Model file for the job. Use its own axes, mm. Round coordinates to 2 decimals unless told otherwise and drop trailing zeros. Order: outer loops, then holes, each group sorted by start corner. A loop starts at its lowest first (then second) coordinate and runs counter-clockwise, first axis right, second up. Notation, with made-up numbers: (-14.75, 75) -> (38.25, 75) arc R22 cw to (38.25, 102) -> close; hole circle Ø4 at (52, 87). An arc over 180 degrees is marked (long way). Answer as CSV lines item,"result".
```python
from build123d import *

# Parameters (mm, degrees)
SKETCH1_W           = 139.7
SKETCH1_H           = 38.1
SKETCH1_R           = 7.1374
BOSS_EXTRUDE1_DEPTH = 4


with BuildPart() as part:
    # Sketch1 → Boss-Extrude1 (new, symmetric)
    with BuildSketch(Plane.XY):
        with Locations((-54.102, 0)):
            Rectangle(SKETCH1_W, SKETCH1_H)
        Circle(SKETCH1_R, mode=Mode.SUBTRACT)
    extrude(amount=BOSS_EXTRUDE1_DEPTH, both=True)


solid = part.part
```
Q1. Saw through at B-B (y = 0). Write the cut outline in (x, z), plus the area to 3 significant figures.
Checks:
outline,"(-123.95, -4) -> (-7.14, -4) -> (-7.14, 4) -> (-123.95, 4) -> close; (7.14, -4) -> (15.75, -4) -> (15.75, 4) -> (7.14, 4) -> close"
area,"1,000 mm²"
Q2. Saw through at A-A (x = 0). Write the cut outline in (y, z).
Checks:
outline,"(-19.05, -4) -> (-7.14, -4) -> (-7.14, 4) -> (-19.05, 4) -> close; (7.14, -4) -> (19.05, -4) -> (19.05, 4) -> (7.14, 4) -> close"
Q3. Wall check: L1, parallel to Y at x = 0, z = -0.75; L2, parallel to X at y = -0.5, z = -3.25; L3, parallel to X at y = 5, z = -1.25. Give the ranges that are in metal, low to high. Write a range as [from, to].
Checks:
L1,"[-19.05, -7.14], [7.14, 19.05]"
L2,"[-123.95, -7.12], [7.12, 15.75]"
L3,"[-123.95, -5.09], [5.09, 15.75]"
Q4. Mould opens along Y. For faces 1 (the flat face through (-55, 19.05, 0)), 2 (the flat face through (-55, 0, 4)), 3 (the cylindrical face through (-7.13, 0.31, -0.06)) say: +Y half, -Y half, draft (parallel to the pull), parting line (faces both ways), or undercut.
Checks:
face 1,"+Y half"
face 2,"draft"
face 3,"undercut"
Q5. Saw through at C-C (z = 2.75). Write the cut outline in (x, y), plus the area to 3 significant figures.
Checks:
outline,"(-123.95, -19.05) -> (15.75, -19.05) -> (15.75, 19.05) -> (-123.95, 19.05) -> close; hole circle Ø14.27 at (0, 0)"
area,"5,160 mm²"
